from build123d import *

# Parameters (mm, degrees)
SKETCH1_W           = 16
SKETCH1_H           = 10
BOSS_EXTRUDE1_DEPTH = 6
M6_TAPPED_HOLE1_D   = 5


with BuildPart() as part:
    # Sketch1 → Boss-Extrude1 (new body)
    with BuildSketch(Plane.XY):
        Rectangle(SKETCH1_W, SKETCH1_H)
    extrude(amount=BOSS_EXTRUDE1_DEPTH)

    # M6 Tapped Hole1 (through all)
    with Locations(Plane.XY.offset(6)):
        with Locations((0, 0)):
            Hole(M6_TAPPED_HOLE1_D / 2)


solid = part.part
Here's how the part is built. I have some questions about the finished solid (model axes, mm). Coordinates: 2 decimals unless noted, no trailing zeros. Order: outer loops, then holes, each group sorted by start corner. A loop starts at its lowest first (then second) coordinate and runs counter-clockwise, first axis right, second up. Notation, with made-up numbers: (45.5, 8) - (101.5, 8) arc R34 ccw to (101.5, 38) - close; hole circle Ø1 at (87, 82.25). An arc over 180 degrees is marked (long way). Use CSV: the item, a comma, the result in double quotes. Start each with the question number.
1. Please list where these lines run through material, in increasing order: line 1 (Y direction, x = 0, z = 2.9); line 2 (X direction, y = -2, z = 4); line 3 (X direction, y = 0.5, z = 2.4). Write a range as from..to.
2. I'm going to push flat-ended pins straight in: pin 1 (3 mm diameter, centred on x = -4.5, y = -1.5, fed in from -Z); pin 2 (4.5 mm diameter, centred on x = 0, y = 0, fed in from -Z). Where does each tip first touch, or does it pass through?
3. If we mould it in two halves opening along Y, with no side actions, what happens to faces 1 (the face through (8, 0, 3)), 2 (the face through (0.54, -2.44, 2.96)), 3 (the face through (0, -5, 3)), 4 (the face through (0, 5, 3))? For each: +Y half, -Y half, draft (parallel to the pull), parting line (faces both ways), or undercut.
4. Suppose I cut it at C-C on z = 2.65. List the corners of the cut face in (x, y) for me, then the cut area to 3 significant figures.
5. Suppose I cut it at A-A on y = 0. List the corners of the cut face in (x, z) for me, then the cut area to 3 significant figures.
6. Suppose I cut it at B-B on x = 1.5. List the corners of the cut face in (y, z) for me.
Output:
1,line 1,"y = -5..-2.5, 2.5..5"
1,line 2,"x = -8..-1.5, 1.5..8"
1,line 3,"x = -8..-2.45, 2.45..8"
2,pin 1,"stops at z = 0"
2,pin 2,"passes through"
3,face 1,"draft"
3,face 2,"undercut"
3,face 3,"-Y half"
3,face 4,"+Y half"
4,outline,"(-8, -5) - (8, -5) - (8, 5) - (-8, 5) - close; hole circle Ø5 at (0, 0)"
4,area,"140 mm2"
5,outline,"(-8, 0) - (-2.5, 0) - (-2.5, 6) - (-8, 6) - close; (2.5, 0) - (8, 0) - (8, 6) - (2.5, 6) - close"
5,area,"66.0 mm2"
6,outline,"(-5, 0) - (-2, 0) - (-2, 6) - (-5, 6) - close; (2, 0) - (5, 0) - (5, 6) - (2, 6) - close"
